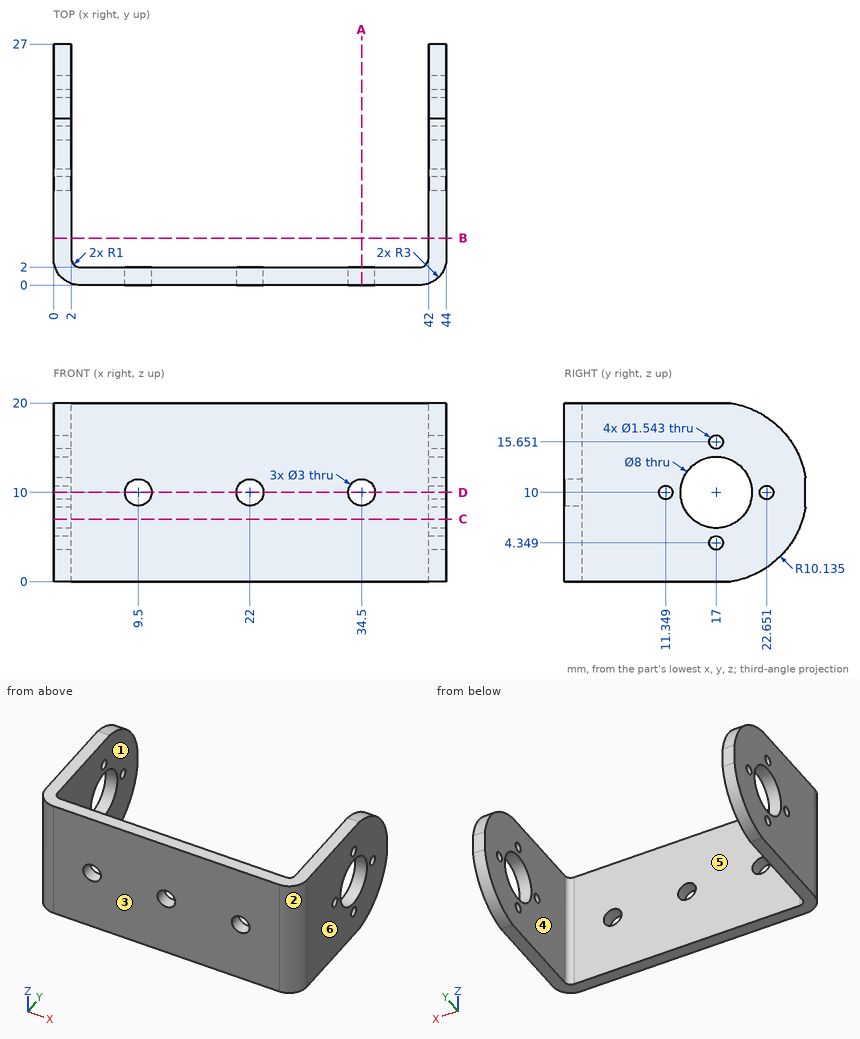
Input: dimensioned drawing with shaded views. Units: mm. Origin: part minimum x, y, z. A direction names the side the tool comes from. Coordinates: 2 decimals unless noted, no trailing zeros. Order: outer loops, then holes, each group sorted by start corner. A loop starts at its lowest first (then second) coordinate and runs counter-clockwise, first axis right, second up.
(1) Access query for the marked faces 5 and 6. Directions: +Z, -Z, +X, -X, +Y, -Y. A direction counts if a zero-diameter tool reaches every point of the face in a straight line with its end or side. Return the directions, or none.
(2) Section query A-A (x = 34.5). Return the cut outline in (y, z).
(3) Section query B-B (y = 5.25). Return the cut outline in (x, z).
(4) First-contact query: pin 1 (1.8 mm diameter, centred on y = 11.35, z = 10, fed in from +X); pin 2 (6 mm diameter, centred on x = 14.5, z = 7, fed in from +Y). Flat tips, straight axial feed; report the tip coordinate or a pass-through.
(5) Section query D-D (z = 10). State how many separate pieces and enclosed holes the cut face has, plus the area to 3 significant figures.
(6) Section query C-C (z = 7). Return the cut outline in (x, y) (1 decimal).
(7) Material intervals for probe 1 along X at (y, z) = (19.25, 13.5); probe 2 along X at (y, z) = (1.25, 10) (1 decimal); probe 3 along Y at (x, z) = (42.55, 10), sorted ascending.
(8) Draft query along X for the marked faces 1, 2, 3 and 4. Return one class per face: pulls with the +X half, pulls with the -X half, needs draft (parallel to the pull), parting line crosses it, or undercut.
Solution:
1. face 5: +Z, -Z, +Y
1. face 6: +Z, -Z, +X, +Y, -Y
2. outline: (0, 0) - (2, 0) - (2, 8.5) - (0, 8.5) - close; (0, 11.5) - (2, 11.5) - (2, 20) - (0, 20) - close
3. outline: (0, 0) - (2, 0) - (2, 20) - (0, 20) - close; (42, 0) - (44, 0) - (44, 20) - (42, 20) - close
4. pin 1: stops at x = 44
4. pin 2: stops at y = 2
5. separate pieces: 10
5. enclosed holes: 0
5. area: 122 mm2
6. outline: (0, 3) arc R3 ccw to (3, 0) - (41, 0) arc R3 ccw to (44, 3) - (44, 14.4) - (42, 14.4) - (42, 3) arc R1 cw to (41, 2) - (3, 2) arc R1 cw to (2, 3) - (2, 14.4) - (0, 14.4) - close; (0, 19.6) - (2, 19.6) - (2, 26.7) - (0, 26.7) - close; (42, 19.6) - (44, 19.6) - (44, 26.7) - (42, 26.7) - close
7. probe 1: x = 0 to 2, 42 to 44
7. probe 2: x = 0.6 to 8, 11 to 20.5, 23.5 to 33, 36 to 43.4
7. probe 3: y = 0.43 to 10.58, 12.12 to 13, 21 to 21.88, 23.42 to 27
8. face 1: undercut
8. face 2: pulls with the +X half
8. face 3: needs draft
8. face 4: undercut
